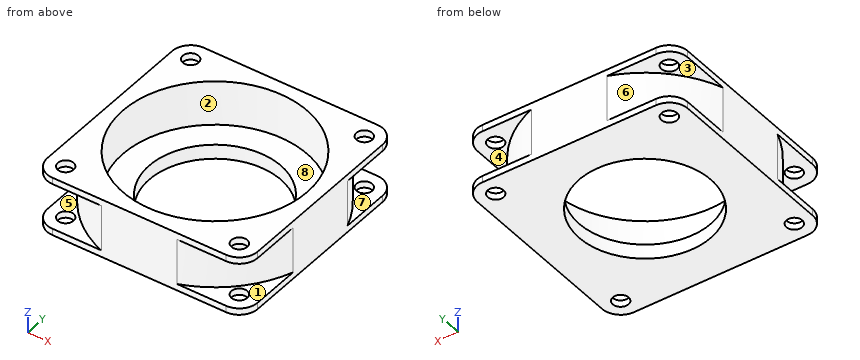
from build123d import *

# Parameters (mm, degrees)
FRONT_FLANGE_80X80_DEPTH = 2.5
HUB_SKETCH_R             = 35
HUB_70_DEPTH             = 20
REAR_START               = -2.5
REAR_FLANGE_80X80_DEPTH  = 2.5
SIDE_WEBS_DEPTH          = 20
LARGE_BORE_SKETCH_R      = 35
LARGE_BORE_70_DEPTH      = 17
THROUGH_BORE_SKETCH_R    = 25
THROUGH_BORE_50_DEPTH    = 8
CORNER_HOLES_SKETCH_R    = 3
CORNER_HOLES_4X_6_DEPTH  = 25


with BuildPart() as part:
    # Front Flange Sketch → Front Flange 80x80 (new body)
    with BuildSketch(Plane.XY):
        with BuildLine():
            Line((0, 0), (33, 0))
            ThreePointArc((33, 0), (37.949747468, 2.050252532), (40, 7))
            Line((40, 7), (40, 73))
            ThreePointArc((40, 73), (37.949747468, 77.949747468), (33, 80))
            Line((33, 80), (-33, 80))
            ThreePointArc((-33, 80), (-37.949747468, 77.949747468), (-40, 73))
            Line((-40, 73), (-40, 7))
            ThreePointArc((-40, 7), (-37.949747468, 2.050252532), (-33, 0))
            Line((-33, 0), (0, 0))
        make_face()
    extrude(amount=FRONT_FLANGE_80X80_DEPTH)

    # Hub Sketch → Hub Ø70 (add)
    with BuildSketch(Plane.XY.offset(2.5)):
        with Locations((0, 40)):
            Circle(HUB_SKETCH_R)
    extrude(amount=HUB_70_DEPTH)

    # Rear Flange Sketch → Rear Flange 80x80 (add)
    with BuildSketch(Plane.XY.offset(22.5).offset(REAR_START)):
        with BuildLine():
            Line((40, 7), (40, 40))
            Line((40, 40), (40, 73))
            ThreePointArc((40, 73), (37.949747468, 77.949747468), (33, 80))
            Line((33, 80), (-33, 80))
            ThreePointArc((-33, 80), (-37.949747468, 77.949747468), (-40, 73))
            Line((-40, 73), (-40, 7))
            ThreePointArc((-40, 7), (-37.949747468, 2.050252532), (-33, 0))
            Line((-33, 0), (33, 0))
            ThreePointArc((33, 0), (37.949747468, 2.050252532), (40, 7))
        make_face()
    extrude(amount=REAR_FLANGE_80X80_DEPTH)

    # Side Web Sketch → Side Webs (add)
    with BuildSketch(Plane.XY.offset(22.5)):
        with BuildLine():
            Line((-14.361406616, 80), (14.361406616, 80))
            ThreePointArc((14.361406616, 80), (30.0520382, 70.0520382), (40, 54.361406616))
            Line((40, 54.361406616), (40, 25.638593384))
            ThreePointArc((40, 25.638593384), (30.0520382, 9.9479618), (14.361406616, 0))
            Line((14.361406616, 0), (-14.361406616, 0))
            ThreePointArc((-14.361406616, 0), (-30.0520382, 9.9479618), (-40, 25.638593384))
            Line((-40, 25.638593384), (-40, 54.361406616))
            ThreePointArc((-40, 54.361406616), (-30.0520382, 70.0520382), (-14.361406616, 80))
        make_face()
    extrude(amount=-SIDE_WEBS_DEPTH)

    # Large Bore Sketch → Large Bore Ø70 (cut)
    with BuildSketch(Plane.XY.offset(22.5)):
        with Locations((0, 40)):
            Circle(LARGE_BORE_SKETCH_R)
    extrude(amount=-LARGE_BORE_70_DEPTH, mode=Mode.SUBTRACT)

    # Through Bore Sketch → Through Bore Ø50 (cut)
    with BuildSketch(Plane.XY.offset(5.5)):
        with Locations((0, 40)):
            Circle(THROUGH_BORE_SKETCH_R)
    extrude(amount=-THROUGH_BORE_50_DEPTH, mode=Mode.SUBTRACT)

    # Corner Holes Sketch → Corner Holes 4xØ6 (cut)
    with BuildSketch(Plane.XY.offset(22.5)):
        with Locations((-33, 73)):
            Circle(CORNER_HOLES_SKETCH_R)
        with Locations((33, 73)):
            Circle(CORNER_HOLES_SKETCH_R)
        with Locations((-33, 7)):
            Circle(CORNER_HOLES_SKETCH_R)
        with Locations((33, 7)):
            Circle(CORNER_HOLES_SKETCH_R)
    extrude(amount=-CORNER_HOLES_4X_6_DEPTH, mode=Mode.SUBTRACT)


solid = part.part
For this review, take the finished solid that the model builds, in its own axes (mm). Face numbers are marked on the shaded views. A direction names the side the tool comes from. Round coordinates to 2 decimals unless told otherwise and drop trailing zeros. Write each loop counter-clockwise with the first axis right and the second up, starting at its lowest first coordinate (ties: lowest second). Pieces come first, ordered by that corner, then holes. Notation, with made-up numbers: (75.5, -38) -> (123.5, -38) arc R19 ccw to (123.5, -27) -> close; hole circle Ø7 at (56.25, -23.5). An arc over 180 degrees is marked (long way). Use CSV: the item, a comma, the result in double quotes.
(1) Consider section B-B, the plane y = 40. Give the boundary of the cut face in (x, z).
Computed values:
outline,"(-40, 0) -> (-25, 0) -> (-25, 5.5) -> (-35, 5.5) -> (-35, 22.5) -> (-40, 22.5) -> close; (25, 0) -> (40, 0) -> (40, 22.5) -> (35, 22.5) -> (35, 5.5) -> (25, 5.5) -> close"
(2) Consider section A-A, the plane x = 0. Give the boundary of the cut face in (y, z).
Computed values:
outline,"(0, 0) -> (15, 0) -> (15, 5.5) -> (5, 5.5) -> (5, 22.5) -> (0, 22.5) -> close; (65, 0) -> (80, 0) -> (80, 22.5) -> (75, 22.5) -> (75, 5.5) -> (65, 5.5) -> close"
(3) For the marked faces 1, 2, 3, 4 and 5, list the 3-axis set-ups (+Z, -Z, +X, -X, +Y, -Y) from which the entire face can be reached by the end or side of a thin tool; tool diameter is ignored.
Computed values:
face 1,"+X, -Y"
face 2,"+Z"
face 3,"-X, +Y"
face 4,"+X, +Y"
face 5,"-X, -Y"
(4) Consider section C-C, the plane z = 18. Give the boundary of the cut face in (x, y).
Computed values:
outline,"(-40, 25.64) arc R42.5 ccw to (-14.36, 0) -> (14.36, 0) arc R42.5 ccw to (40, 25.64) -> (40, 54.36) arc R42.5 ccw to (14.36, 80) -> (-14.36, 80) arc R42.5 ccw to (-40, 54.36) -> close; hole circle Ø70 at (0, 40)"
(5) Clearance check with flat-ended pins moving along their axes: P1, Ø5.5, axis at x = -33, y = 73, coming from the -Z side; P2, Ø1.5, axis at x = -17.5, z = 9.5, coming from the +Y side; P3, Ø1, axis at x = 23, z = 15, coming from the -Y side; P4, Ø1, axis at x = 15.5, z = 17.5, coming from the +Y side. State where each tip first meets the part, or that it passes through.
Computed values:
P1,"through"
P2,"y = 79.06"
P3,"y = 3.94"
P4,"y = 79.76"
(6) Consider section D-D, the plane x = 29. Give the boundary of the cut face in (y, z), plus the area to 3 significant figures.
Computed values:
outline,"(0, 0) -> (80, 0) -> (80, 2.5) -> (71.07, 2.5) -> (71.07, 20) -> (80, 20) -> (80, 22.5) -> (59.6, 22.5) -> (59.6, 5.5) -> (20.4, 5.5) -> (20.4, 22.5) -> (0, 22.5) -> (0, 20) -> (8.93, 20) -> (8.93, 2.5) -> (0, 2.5) -> close"
area,"821 mm²"
(7) To check wall thickness, follow L1, parallel to Z at x = -31, y = 76.5; L2, parallel to X at y = 63, z = 1.25; L3, parallel to X at y = 58, z = 6.75. State the ranges of each line that lie inside material, in increasing order. Write a range as [from, to].
Computed values:
L1,"[0, 2.5], [20, 22.5]"
L2,"[-40, -9.8], [9.8, 40]"
L3,"[-38.5, -30.02], [30.02, 38.5]"
(8) Draft analysis for pull direction Y (two halves, no side actions). For the marked faces 6, 7 and 8, state which applies: +Y half, -Y half, draft (parallel to the pull), parting line (faces both ways), or undercut.
Computed values:
face 6,"+Y half"
face 7,"draft"
face 8,"undercut"
